Could you check a few things on this model? Use its own coordinates, in mm. Coordinates: 2 decimals unless noted, no trailing zeros. Loops run counter-clockwise (first coordinate to the right, second up) from the corner with the lowest first, then second, coordinate; pieces in that order, holes last. Notation, with made-up numbers: M 70.25,-11.5 L 87.25,-11.5 A13 cw 87.25,-3.5 Z; hole C -39.5,18.5 d9. An arc over 180 degrees is marked long. Write each question's results on one line, items separated by ' | '.
```python
from build123d import *

# Parameters (mm, degrees)
SKETCH1_R           = 15
SKETCH1_R_2         = 7.75
BOSS_EXTRUDE1_DEPTH = 10
SKETCH2_W           = 0.1
SKETCH2_H           = 22.468635184
CUT_EXTRUDE1_DEPTH  = 24.452078799


with BuildPart() as part:
    # Sketch1 → Boss-Extrude1 (new body)
    with BuildSketch(Plane.XY):
        Circle(SKETCH1_R)
        Circle(SKETCH1_R_2, mode=Mode.SUBTRACT)
    extrude(amount=BOSS_EXTRUDE1_DEPTH)

    # Sketch2 → Cut-Extrude1 (cut, through all)
    with BuildSketch(Plane.XY.offset(10)):
        with Locations((0, -7.75)):
            Rectangle(SKETCH2_W, SKETCH2_H)
    extrude(amount=-CUT_EXTRUDE1_DEPTH, mode=Mode.SUBTRACT)


solid = part.part
```
(1) Imagine slicing it at B-B, the plane y = -0.5. List the corners of the cut face in (x, z) for me.
Reported:
outline: M -14.99,0 L -7.73,0 L -7.73,10 L -14.99,10 Z; M 7.73,0 L 14.99,0 L 14.99,10 L 7.73,10 Z
(2) Please list where these lines run through material, in increasing order: probe 1 along X at (y, z) = (0, 4.75); probe 2 along Y at (x, z) = (0, 2.75); probe 3 along Y at (x, z) = (6.5, 8.5). Write a range as from..to.
Reported:
probe 1: x = -15..-7.75, 7.75..15 | probe 2: y = 7.75..15 | probe 3: y = -13.52..-4.22, 4.22..13.52
(3) Imagine slicing it at A-A, the plane x = 6.25. List the corners of the cut face in (y, z) for me.
Reported:
outline: M -13.64,0 L -4.58,0 L -4.58,10 L -13.64,10 Z; M 4.58,0 L 13.64,0 L 13.64,10 L 4.58,10 Z
(4) Imagine slicing it at D-D, the plane y = 13.25. List the corners of the cut face in (x, z) for me.
Reported:
outline: M -7.03,0 L 7.03,0 L 7.03,10 L -7.03,10 Z
(5) Imagine slicing it at C-C, the plane z = 4. List the corners of the cut face in (x, y) for me.
Reported:
outline: M -0.05,-15 L -0.05,-7.75 A7.75 cw long 0.05,-7.75 L 0.05,-15 A15 ccw long Z
(6) Will these pins go through, and if not, where does the flat tip stop? P1, Ø1.5, axis at y = -8, z = 7.5, coming from the -X side; P2, Ø2, axis at y = -12, z = 4, coming from the -X side; P3, Ø1, axis at x = -5, z = 2, coming from the -Y side.
Reported:
P1: stops at x = -13.13 | P2: stops at x = -10.2 | P3: stops at y = -14.31
